Can you work these out from the model? Positions are in its coordinate system, mm. Face numbers are marked on the shaded views. Round coordinates to 2 decimals unless told otherwise and drop trailing zeros. Loops run counter-clockwise (first coordinate to the right, second up) from the corner with the lowest first, then second, coordinate; pieces in that order, holes last.
from build123d import *

# Parameters (mm, degrees)
EXTRUDE_1_DEPTH        = 12.5
CUT_EXTRUDE_1_DEPTH    = 1
FILLET_1_R             = 10
FILLET_2_R             = 1
HOLE_WIZARD_M2_1_D     = 1.6
HOLE_WIZARD_M2_1_DEPTH = 5.2
HOLE_WIZARD_M2_1_TIP   = 0.480688495
FILLET_4_R             = 1


with BuildPart() as part:
    # 草图1 → 凸台-拉伸1 (new body)
    with BuildSketch(Plane.XY):
        with BuildLine():
            Line((-7, -7.083005244), (-7, -13.5))
            Line((-7, -13.5), (7, -13.5))
            Line((7, -13.5), (7, 13.5))
            Line((7, 13.5), (-5.417424305, 13.5))
            ThreePointArc((-5.417424305, 13.5), (0.967629177, 2.656726476), (-7, -7.083005244))
        make_face()
    extrude(amount=EXTRUDE_1_DEPTH)

    # 草图2 → 切除-拉伸1 (cut)
    with BuildSketch(Plane(origin=(0, 13.5, 0), x_dir=(1, 0, 0), z_dir=(0, 1, 0))):
        Polygon((-5.417424305, -12.5), (-5.417424305, -8.5), (2, -8.5), (7, -7.5), (7, -12.5), align=None)
    extrude(amount=-CUT_EXTRUDE_1_DEPTH, mode=Mode.SUBTRACT)

    # 圆角1
    fillet_1_edges = [part.edges().sort_by_distance(p)[0] for p in [
        (7, -13.5, 6.25),
    ]]
    fillet(fillet_1_edges, radius=FILLET_1_R)

    # 圆角2
    fillet_2_edges = [part.edges().sort_by_distance(p)[0] for p in [
        (7, 12.5, 10),
    ]]
    fillet(fillet_2_edges, radius=FILLET_2_R)

    # M2 螺纹孔1
    with Locations(Plane(origin=(0, 0, 0), x_dir=(-1, 0, 0), z_dir=(0, 0, -1))):
        with Locations((-4, 2.5), (-4, 10.5)):
            Hole(HOLE_WIZARD_M2_1_D / 2, depth=HOLE_WIZARD_M2_1_DEPTH)
            with Locations((0, 0, -(HOLE_WIZARD_M2_1_DEPTH + HOLE_WIZARD_M2_1_TIP / 2))):  # 118° drill point
                Cone(0, HOLE_WIZARD_M2_1_D / 2, HOLE_WIZARD_M2_1_TIP, mode=Mode.SUBTRACT)

    # 圆角4
    fillet_4_edges = [part.edges().sort_by_distance(p)[0] for p in [
        (-7, -7.083005244, 6.25),
    ]]
    fillet(fillet_4_edges, radius=FILLET_4_R)


solid = part.part
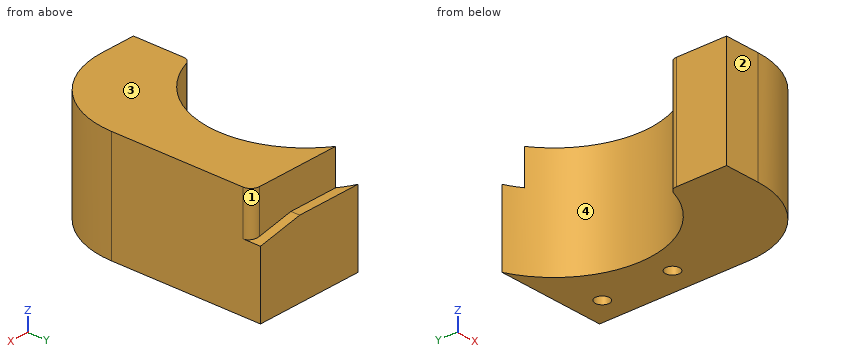
(1) If we section it at C-C, the plane y = -6: List the corners of the cut face in (x, z) for me.
Worked answers:
outline: (-4.45, 0) - (6.68, 0) - (6.68, 12.5) - (-4.45, 12.5) - close
(2) If we section it at A-A, the plane z = 1.5: List the corners of the cut face in (x, y) for me.
Worked answers:
outline: (-7, -13.5) - (-3, -13.5) arc R10 ccw to (7, -3.5) - (7, 13.5) - (-5.42, 13.5) arc R11 cw to (-6.33, -6.87) arc R1 ccw to (-7, -7.81) - close; hole circle Ø1.6 at (4, 2.5); hole circle Ø1.6 at (4, 10.5)
(3) If we section it at B-B, the plane z = 10.25: List the corners of the cut face in (x, y) for me, then the cut area to 3 significant figures.
Worked answers:
outline: (-7, -13.5) - (-3, -13.5) arc R10 ccw to (7, -3.5) - (7, 11.5) arc R1 ccw to (6, 12.5) - (-3.68, 12.5) arc R11 cw to (-6.33, -6.87) arc R1 ccw to (-7, -7.81) - close
area: 220 mm2
(4) Will these pins go through, and if not, where does the flat tip stop? P1, Ø1.4, axis at x = 4, y = 2.5, coming from the -Z side; P2, Ø3, axis at x = 2.5, z = 8, coming from the -Y side; P3, Ø0.5, axis at x = -1, y = 13, coming from the +Z side.
Worked answers:
P1: stops at z = 5.26
P2: stops at y = -12.67
P3: stops at z = 8.5
(5) If we mould it in two halves opening along Y, with no side actions, what happens to the marked faces 1, 2, 3 and 4? For each: released by +Y, released by -Y, zero draft, split by the parting line, or undercut.
Worked answers:
face 1: released by +Y
face 2: released by -Y
face 3: zero draft
face 4: undercut
(6) If we section it at D-D, the plane x = 2.75: List the corners of the cut face in (y, z) for me, then the cut area to 3 significant figures.
Worked answers:
outline: (-11.68, 0) - (13.5, 0) - (13.5, 8.35) - (12.5, 8.35) - (12.5, 12.5) - (-11.68, 12.5) - close
area: 311 mm2
(7) If I drill on line 1 (Y direction, x = 3.75, z = 5.25); line 2 (Y direction, x = 4, z = 2.95); line 3 (Y direction, x = -2, z = 6), over which ranges is the centre line in solid material (lowest first)?
Worked answers:
line 1: y = -10.88 to 1.83, 3.17 to 9.83, 11.17 to 13.5
line 2: y = -10.64 to 1.7, 3.3 to 9.7, 11.3 to 13.5
line 3: y = -13.45 to -4.05, 11.05 to 13.5
